```python
from build123d import *

# Parameters (mm, degrees)
BRACKET_BODY_DEPTH        = 50
THROUGH_HOLE_SKETCH_R     = 10
THROUGH_HOLE_DEPTH        = 50
UPRIGHT_NOTCH_20X10_DEPTH = 15
CORNER_FILLET_R5_R        = 5
SIDE_TAB_DEPTH            = 5


with BuildPart() as part:
    # Bracket L-Profile Sketch → Bracket Body (new body)
    with BuildSketch(Plane.XY):
        Polygon((0, 65), (0, 0), (-30, 0), (-30, 8), (-95, 8), (-95, 16), (-15, 16), (-15, 65), align=None)
    extrude(amount=BRACKET_BODY_DEPTH)

    # Through Hole Sketch → Through Hole (cut)
    with BuildSketch(Plane(origin=(0, 16, 0), x_dir=(1, 0, 0), z_dir=(0, 1, 0))):
        with Locations(Location((-65, -24.700639753, 0), (0, 0, 270))):
            Circle(THROUGH_HOLE_SKETCH_R)
    extrude(amount=-THROUGH_HOLE_DEPTH, mode=Mode.SUBTRACT)

    # Upright Notch Sketch → Upright Notch 20x10 (cut)
    with BuildSketch(Plane(origin=(0, 65, 0), x_dir=(1, 0, 0), z_dir=(0, 1, 0))):
        Polygon((0, -25), (0, -35), (-15, -35), (-15, -15), (0, -15), align=None)
    extrude(amount=-UPRIGHT_NOTCH_20X10_DEPTH, mode=Mode.SUBTRACT)

    # Corner Fillet R5
    corner_fillet_r5_edges = [part.edges().sort_by_distance(p)[0] for p in [
        (-95, 12, 0),
        (-95, 12, 50),
    ]]
    fillet(corner_fillet_r5_edges, radius=CORNER_FILLET_R5_R)

    # Side Tab Sketch → Side Tab (add, symmetric)
    with BuildSketch(Plane(origin=(0, 0, 25), x_dir=(-1, 0, 0), z_dir=(0, 0, -1))):
        Polygon((15, 16), (47, 16), (15, 50), align=None)
    extrude(amount=SIDE_TAB_DEPTH, both=True)


solid = part.part
```
Part model, mm, in its own coordinate system. A direction names the side the tool comes from. Coordinates: 2 decimals unless noted, no trailing zeros. Order: outer loops, then holes, each group sorted by start corner. A loop starts at its lowest first (then second) coordinate and runs counter-clockwise, first axis right, second up. Notation, with made-up numbers: (7, 28.25) -> (51, 28.25) arc R18 cw to (51, 44.25) -> close; hole circle Ø1 at (-4, 16.25). An arc over 180 degrees is marked (long way). Put each result on its own line as item: value. Start each with the question number.
(1) Band-saw the part on C-C (x = -23). Give the cut face in (y, z).
(2) Band-saw the part on A-A (x = -65). Give the cut face in (y, z), then the cut area to 3 significant figures.
(3) Band-saw the part on D-D (y = 25). Give the cut face in (x, z), then the cut area to 3 significant figures.
(4) Pin check, flat tips, straight feed: pin 1 Ø9.5 at (x, y) = (-26.5, 38) entering from -Z; pin 2 Ø6 at (y, z) = (43.5, 13) entering from -X; pin 3 Ø2 at (x, z) = (-74.5, 42) entering from -Y. Stop position of each tip, or through.
(5) Probe line 1 along Y through (x, z) = (-47, 26.5); line 2 along Z through (x, y) = (-20, 31.5); line 3 along X through (y, z) = (3.5, 34). List the from-to ranges inside material, lowest first. Write a range as [from, to].
(6) Band-saw the part on B-B (z = 24). Give the cut face in (x, y).
(7) Mould opens along X. For faces 4 (the face through (-15, 40, 10)), 5 (the face through (-74.76, 12.06, 22.53)), 6 (the face through (-24.8, 15.8, 0)) say: pulls with the +X half, pulls with the -X half, needs draft (parallel to the pull), parting line crosses it, or undercut.
(8) Which spindle directions (+Z, -Z, +X, -X, +Y, -Y) get a long thin tool onto all of the face, cutting with end or side? Do faces 1 (the face through (-54.8, 8, 24.6)), 2 (the face through (-56, 16, 19)), 3 (the face through (-24, 26, 30)). Say none if no direction does.
Determined:
1. outline: (0, 0) -> (16, 0) -> (16, 20) -> (41.5, 20) -> (41.5, 30) -> (16, 30) -> (16, 50) -> (0, 50) -> close
2. outline: (8, 0) -> (16, 0) -> (16, 14.7) -> (8, 14.7) -> close; (8, 34.7) -> (16, 34.7) -> (16, 50) -> (8, 50) -> close
2. area: 240 mm²
3. outline: (-38.53, 20) -> (-15, 20) -> (-15, 0) -> (0, 0) -> (0, 50) -> (-15, 50) -> (-15, 30) -> (-38.53, 30) -> close
3. area: 985 mm²
4. pin 1: stops at z = 20
4. pin 2: stops at x = -15
4. pin 3: stops at y = 8
5. line 1: y = [8, 16]
5. line 2: z = [20, 30]
5. line 3: x = [-30, 0]
6. outline: (-95, 8) -> (-74.98, 8) -> (-74.98, 16) -> (-95, 16) -> close; (-55.02, 8) -> (-30, 8) -> (-30, 0) -> (0, 0) -> (0, 50) -> (-15, 50) -> (-47, 16) -> (-55.02, 16) -> close
7. face 4: pulls with the -X half
7. face 5: undercut
7. face 6: needs draft
8. face 1: +Z, -Z, -X, -Y
8. face 2: -X, +Y
8. face 3: +Z, -X, +Y
